Geometry check sheet. Reference: the model listing, model coordinates, mm. Face numbers are marked on the shaded views. Give positions to 0.01 mm unless a question says otherwise; leave off trailing zeros. Loops run counter-clockwise (first coordinate to the right, second up) from the corner with the lowest first, then second, coordinate; pieces in that order, holes last. Notation, with made-up numbers: (22.25, 52) -> (35.25, 52) arc R8 ccw to (35.25, 61) -> close; hole circle Ø11 at (-25.75, 28.25). An arc over 180 degrees is marked (long way). Write item = value, one per line.
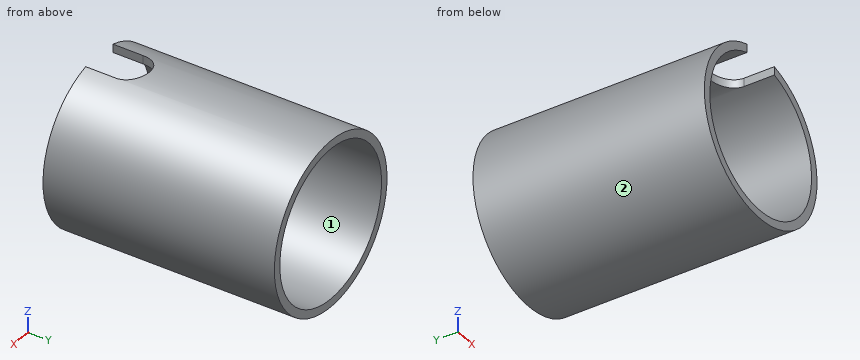
```python
from build123d import *

# Parameters (mm, degrees)
SKETCH1_R               = 82.5
SKETCH1_R_2             = 74.5
BOSS_EXTRUDE1_DEPTH     = 230
CUT_EXTRUDE1_REACH      = 259.9
CUT_EXTRUDE1_END_RADIUS = 82.5


with BuildPart() as part:
    # Sketch1 → Boss-Extrude1 (new body)
    with BuildSketch(Plane(origin=(0, 0, 0), x_dir=(1, 0, 0), z_dir=(0, 1, 0))):
        with Locations(Location((0, 0, 0), (0, 0, 270))):
            Circle(SKETCH1_R)
        with Locations(Location((0, 0, 0), (0, 0, 270))):
            Circle(SKETCH1_R_2, mode=Mode.SUBTRACT)
    extrude(amount=BOSS_EXTRUDE1_DEPTH)

    # Cut-Extrude1: up to this cylinder (the profile starts inside it)
    cut_extrude1_end = Plane(origin=(0, 15, 0), z_dir=(0, -1, 0)) * Cylinder(CUT_EXTRUDE1_END_RADIUS, 685.8, mode=Mode.PRIVATE)
    # Sketch2 → Cut-Extrude1 (cut, up to the surface)
    with BuildSketch(Plane.XY, mode=Mode.PRIVATE) as cut_extrude1_sk1:
        with BuildLine():
            Line((-20, 0), (-20, 30))
            ThreePointArc((-20, 30), (0, 50), (20, 30))
            Line((20, 30), (20, 0))
            ThreePointArc((20, 0), (0, -20), (-20, 0))
        make_face()
    cut_extrude1_tool1 = extrude(cut_extrude1_sk1.sketch, amount=CUT_EXTRUDE1_REACH, mode=Mode.PRIVATE) & cut_extrude1_end
    add(cut_extrude1_tool1.solids().sort_by_distance((0, 15, 0))[0], mode=Mode.SUBTRACT)


solid = part.part
```
Item 1: Section check A-A, the plane z = 0. Record the cut outline in (x, y), plus the area to 3 significant figures.
Answer:
outline = (-82.5, 0) -> (-74.5, 0) -> (-74.5, 230) -> (-82.5, 230) -> close; (74.5, 0) -> (82.5, 0) -> (82.5, 230) -> (74.5, 230) -> close
area = 3,680 mm^2
Item 2: Section check C-C, the plane y = 136. Record the cut outline in (x, z), plus the area to 3 significant figures.
Answer:
outline = circle Ø165 at (0, 0); hole circle Ø149 at (0, 0)
area = 3,950 mm^2
Item 3: Gauge pin test, flat ends, axial feed: pin 1 (4 mm diameter, centred on x = -30, y = 52, fed in from +Z); pin 2 (9 mm diameter, centred on y = 15.5, z = 76.5, fed in from -X); pin 3 (12 mm diameter, centred on y = 146, z = 46.5, fed in from +X). Record the tip position at first contact, or that the pin passes through.
Answer:
pin_1 = 77.6
pin_2 = -40.28
pin_3 = 71.87
Item 4: Section check B-B, the plane x = 23. Record the cut outline in (y, z).
Answer:
outline = (0, -79.23) -> (230, -79.23) -> (230, -70.86) -> (0, -70.86) -> close; (0, 70.86) -> (230, 70.86) -> (230, 79.23) -> (0, 79.23) -> close
Item 5: Draft check along X on the marked faces 1 and 2. Enter one of: +X half, -X half, draft (parallel to the pull), parting line (faces both ways), or undercut.
Answer:
face_1 = undercut
face_2 = parting line
Item 6: Thickness scan on L1, parallel to X at y = 61.5, z = 0; L2, parallel to Z at x = -26.5, y = 44.5; L3, parallel to Z at x = 27, y = 216.5. Record the ranges inside material, lowest first. Write a range as [from, to].
Answer:
L1 = [-82.5, -74.5], [74.5, 82.5]
L2 = [-78.13, -69.63], [69.63, 78.13]
L3 = [-77.96, -69.44], [69.44, 77.96]
